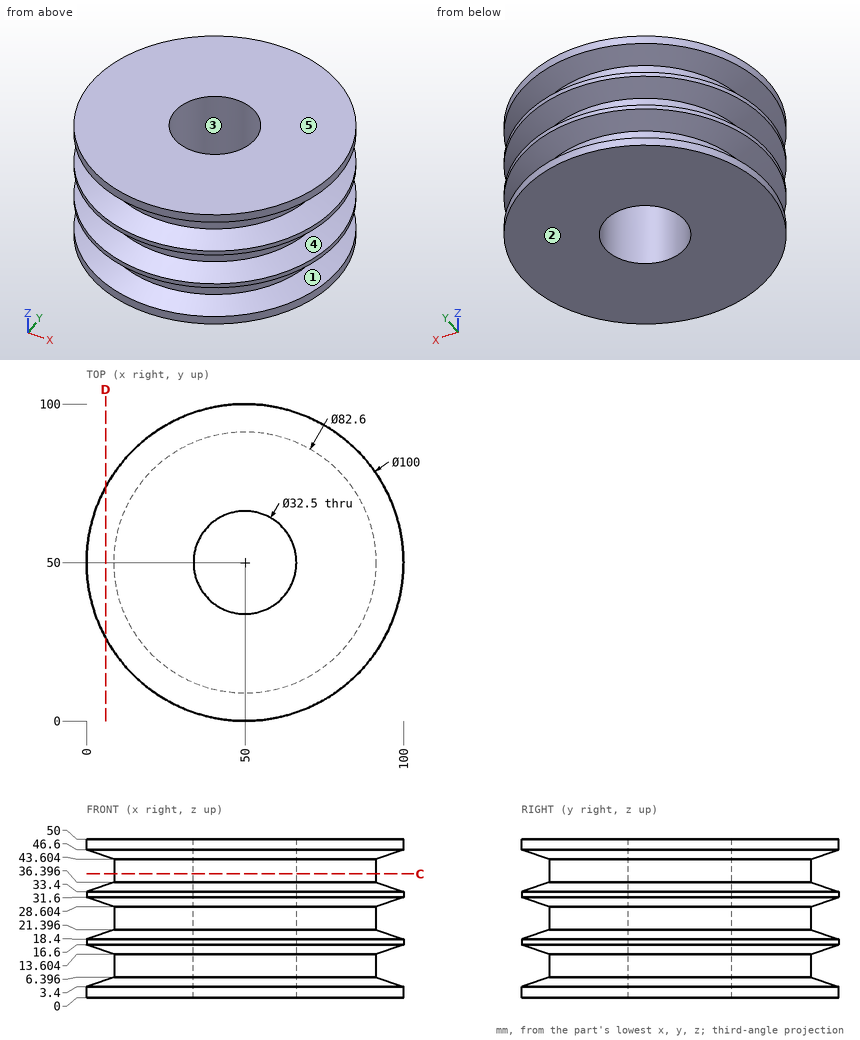
Verification items for this drawing (mm, ordinates from the low corner). A direction names the side the tool comes from. Give positions to 0.01 mm unless a question says otherwise; leave off trailing zeros. Order: outer loops, then holes, each group sorted by start corner. A loop starts at its lowest first (then second) coordinate and runs counter-clockwise, first axis right, second up. Notation, with made-up numbers: M 74,-40 L 90,-40 A22 cw 90,-9 Z; hole C 81.5,45 d9. An arc over 180 degrees is marked long. Use a Markdown table: item, result.
Item 1: Tool access check on the marked faces 4 and 5. Record the directions out of +Z, -Z, +X, -X, +Y, -Y that give a thin tool (end or side, any length) a straight path to the whole face; none if there is none.
Answers follow:
| item | result |
|---|---|
| face 4 | none |
| face 5 | +Z, +X, -X, +Y, -Y |
Item 2: Section check D-D (x = 6). State how many separate pieces and enclosed holes the cut face has.
Answers follow:
| item | result |
|---|---|
| separate pieces | 4 |
| enclosed holes | 0 |
Item 3: Section check C-C (z = 39). Record the cut outline in (x, y).
Answers follow:
| item | result |
|---|---|
| outline | C 50,50 d82.6; hole C 50,50 d32.5 |
Item 4: Material ranges on line 1 along Y through (x, z) = (50, 37.5); line 2 along Z through (x, y) = (79.5, 12); line 3 along Z through (x, y) = (33, 6) (1 decimal), recorded low to high.
Answers follow:
| item | result |
|---|---|
| line 1 | y = 8.7 to 33.75, 66.25 to 91.3 |
| line 2 | z = 0 to 4.05, 15.95 to 19.05, 30.95 to 34.05, 45.95 to 50 |
| line 3 | z = 0 to 4.4, 15.6 to 19.4, 30.6 to 34.4, 45.6 to 50 |
Item 5: Draft check along X on the marked faces 1, 2 and 3. Enter one of: +X half, -X half, draft (parallel to the pull), parting line (faces both ways), or undercut.
Answers follow:
| item | result |
|---|---|
| face 1 | parting line |
| face 2 | draft |
| face 3 | undercut |
Item 6: Depth check by flat-ended pin: P1, Ø10, axis at x = 30, y = 71, coming from the -Z side; P2, Ø1, axis at x = 77, z = 18.5, coming from the +Y side; P3, Ø2, axis at x = 78, z = 38.5, coming from the -Y side; P4, Ø1.5, axis at y = 15, z = 27, coming from the -X side. Enter the tip coordinate at first touch or a pass-through.
Answers follow:
| item | result |
|---|---|
| P1 | stops at z = 0 |
| P2 | stops at y = 92.39 |
| P3 | stops at y = 18.75 |
| P4 | stops at x = 26.92 |
